Job drawing, mm, ordinate dimensions from the low corner. One solid piece. A direction names the side the tool comes from. Round coordinates to 2 decimals unless told otherwise and drop trailing zeros. Loops run counter-clockwise (first coordinate to the right, second up) from the corner with the lowest first, then second, coordinate; pieces in that order, holes last. Notation, with made-up numbers: M 30.5,-31 L 45.5,-31 A24 ccw 45.5,-12 Z; hole C 11,-7 d3. An arc over 180 degrees is marked long. Put each result on its own line as item: value. Start each with the question number.
1) Which spindle directions (+Z, -Z, +X, -X, +Y, -Y) get a long thin tool onto all of the face, cutting with end or side? Do the marked faces 5 and 6. Say none if no direction does.
2) Pull direction Y, two halves, no side cores. Call the marked faces 1, 2, 3 and 4: +Y half, -Y half, draft (parallel to the pull), parting line (faces both ways), or undercut.
3) Slice it at D-D on z = 2.5. Give the cut face in (x, y), then the cut area to 3 significant figures.
4) Drop a flat-ended pin along its axis: pin 1 Ø2 at (x, y) = (25.25, 5) entering from +Z. Give the stop position or say it passes through.
5) Probe line 1 along Y through (x, z) = (25.25, 5.25); line 2 along Y through (x, z) = (4.75, 1.35); line 3 along X through (y, z) = (4, 6.75). List the from-to ranges inside material, lowest first.
6) Slice it at B-B on y = 5. Give the cut face in (x, z), then the cut area to 3 significant figures.
7) Slice it at A-A on x = 25.25. Give the cut face in (y, z).
8) Slice it at C-C on z = 6.5. Give the cut face in (x, y), then the cut area to 3 significant figures.
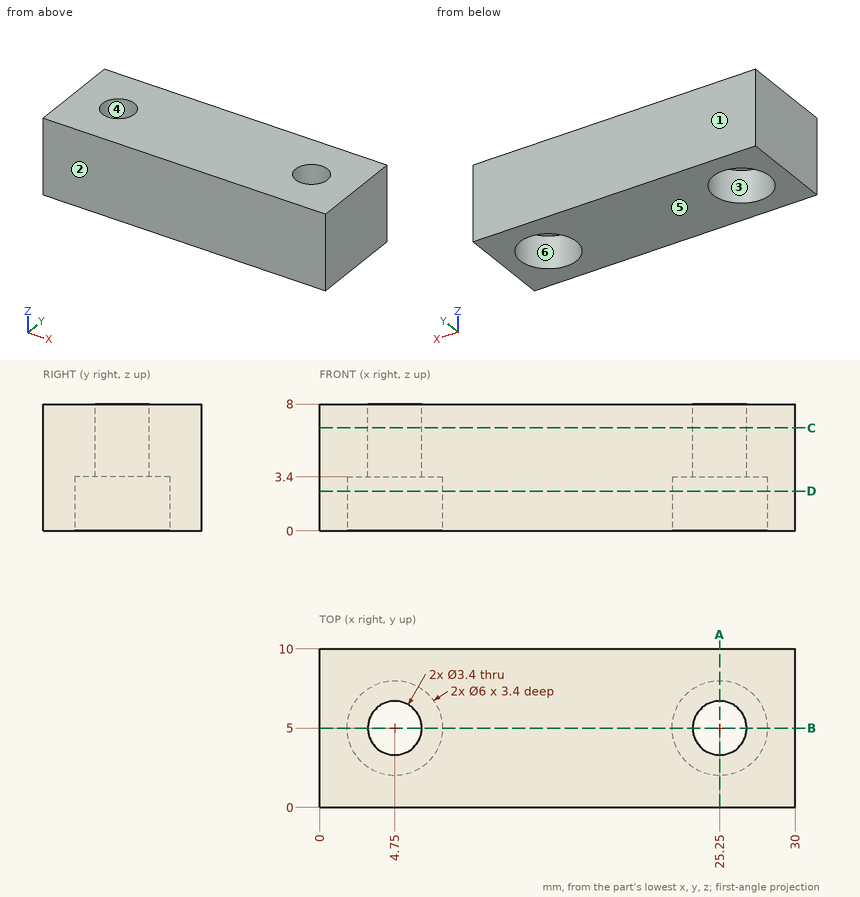
Recorded:
1. face 5: -Z, +X, -X, +Y, -Y
1. face 6: -Z
2. face 1: +Y half
2. face 2: -Y half
2. face 3: undercut
2. face 4: undercut
3. outline: M 0,0 L 30,0 L 30,10 L 0,10 Z; hole C 4.75,5 d6; hole C 25.25,5 d6
3. area: 243 mm2
4. pin 1: passes through
5. line 1: y = 0 to 3.3, 6.7 to 10
5. line 2: y = 0 to 2, 8 to 10
5. line 3: x = 0 to 3.38, 6.12 to 23.88, 26.62 to 30
6. outline: M 0,0 L 1.75,0 L 1.75,3.4 L 3.05,3.4 L 3.05,8 L 0,8 Z; M 6.45,3.4 L 7.75,3.4 L 7.75,0 L 22.25,0 L 22.25,3.4 L 23.55,3.4 L 23.55,8 L 6.45,8 Z; M 26.95,3.4 L 28.25,3.4 L 28.25,0 L 30,0 L 30,8 L 26.95,8 Z
6. area: 168 mm2
7. outline: M 0,0 L 2,0 L 2,3.4 L 3.3,3.4 L 3.3,8 L 0,8 Z; M 6.7,3.4 L 8,3.4 L 8,0 L 10,0 L 10,8 L 6.7,8 Z
8. outline: M 0,0 L 30,0 L 30,10 L 0,10 Z; hole C 4.75,5 d3.4; hole C 25.25,5 d3.4
8. area: 282 mm2
